Drawing for the job (mm, zero at the part's lowest x, y, z). A direction names the side the tool comes from. Round coordinates to 2 decimals unless told otherwise and drop trailing zeros. Loops run counter-clockwise (first coordinate to the right, second up) from the corner with the lowest first, then second, coordinate; pieces in that order, holes last. Notation, with made-up numbers: M -6.75,74.5 L 13.25,74.5 A9 ccw 13.25,89.5 Z; hole C 20.25,60.5 d9. An arc over 180 degrees is marked long. Answer in a Markdown table with one row per item.
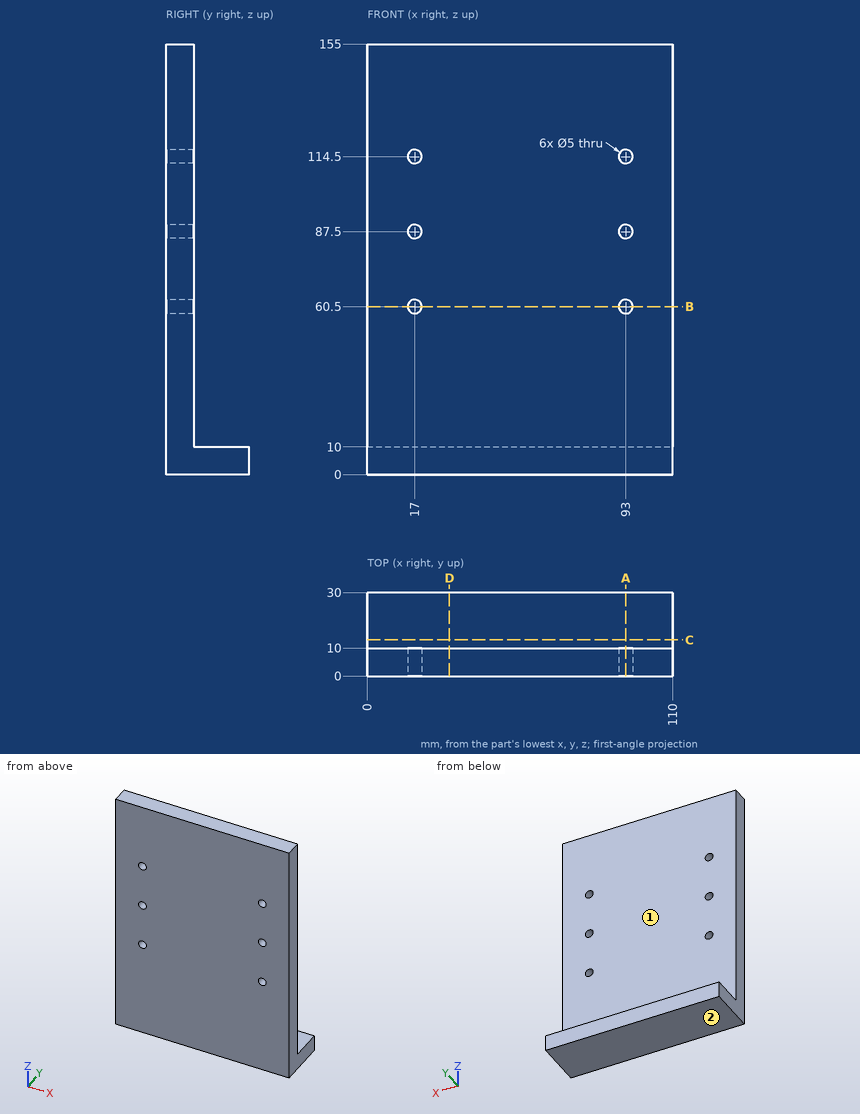
1. Saw through at B-B (z = 60.5). Write the cut outline in (x, y).
Verdict:
| item | result |
|---|---|
| outline | M 0,0 L 14.5,0 L 14.5,10 L 0,10 Z; M 19.5,0 L 90.5,0 L 90.5,10 L 19.5,10 Z; M 95.5,0 L 110,0 L 110,10 L 95.5,10 Z |
2. Saw through at A-A (x = 93). Write the cut outline in (y, z), and give its area (3 significant figures).
Verdict:
| item | result |
|---|---|
| outline | M 0,0 L 30,0 L 30,10 L 10,10 L 10,58 L 0,58 Z; M 0,63 L 10,63 L 10,85 L 0,85 Z; M 0,90 L 10,90 L 10,112 L 0,112 Z; M 0,117 L 10,117 L 10,155 L 0,155 Z |
| area | 1,600 mm² |
3. Pin check, flat tips, straight feed: pin 1 (2 mm diameter, centred on x = 87, y = 17, fed in from +Z); pin 2 (3 mm diameter, centred on x = 17, z = 114.5, fed in from +Y); pin 3 (5 mm diameter, centred on x = 92.5, z = 59.5, fed in from +Y). Stop position of each tip, or through.
Verdict:
| item | result |
|---|---|
| pin 1 | stops at z = 10 |
| pin 2 | passes through |
| pin 3 | stops at y = 10 |
4. Tool access for the marked faces 1 and 2: list every direction of +Z, -Z, +X, -X, +Y, -Y with a clear straight run to the whole face (end or side of a thin tool).
Verdict:
| item | result |
|---|---|
| face 1 | +Z, +X, -X, +Y |
| face 2 | -Z, +X, -X, +Y, -Y |
5. Wall check: probe 1 along Z at (x, y) = (17, 4.5); probe 2 along X at (y, z) = (6.5, 87.5); probe 3 along Y at (x, z) = (75, 57.5). Give the ranges that are in metal, low to high.
Verdict:
| item | result |
|---|---|
| probe 1 | z = 0 to 58, 63 to 85, 90 to 112, 117 to 155 |
| probe 2 | x = 0 to 14.5, 19.5 to 90.5, 95.5 to 110 |
| probe 3 | y = 0 to 10 |
6. Saw through at C-C (y = 13). Write the cut outline in (x, z), and give its area (3 significant figures).
Verdict:
| item | result |
|---|---|
| outline | M 0,0 L 110,0 L 110,10 L 0,10 Z |
| area | 1,100 mm² |
7. Saw through at D-D (x = 29.5). Write the cut outline in (y, z).
Verdict:
| item | result |
|---|---|
| outline | M 0,0 L 30,0 L 30,10 L 10,10 L 10,155 L 0,155 Z |
